Work out the finished part from the listing and answer in its coordinate system (mm). Coordinates: 2 decimals unless noted, no trailing zeros. Loops run counter-clockwise (first coordinate to the right, second up) from the corner with the lowest first, then second, coordinate; pieces in that order, holes last. Notation, with made-up numbers: (-25, -8.75) - (1, -8.75) arc R21 ccw to (1, 21.25) - close; hole circle Ø7 at (-28, 4.25). An arc over 180 degrees is marked (long way). Write each question's results on one line, items separated by ' | '. Start each with the question number.
1. Find the intervals of material crossed by line 1 along X through (y, z) = (2, 2.75); line 2 along Y through (x, z) = (-1.5, 4.1); line 3 along X through (y, z) = (-1.75, 0.8), in increasing order. Write a range as [from, to].
2. Each of these flat-tipped pins is pushed along its axis until it touches: P1, Ø1.5, axis at x = -3, z = 1, coming from the -Y side; P2, Ø2, axis at y = 0.5, z = 2.5, coming from the +X side (3 decimals); P3, Ø3, axis at y = 0, z = 2, coming from the -X side (3 decimals); P4, Ø4, axis at x = 0, y = 0, coming from the -Z side. Where does it stop, or does it pass through?
3. Determine the mould class of faces 1 (the flat face through (3.221, -1.895, 2.761)), 2 (the conical face through (-1.978, -3.406, 5.546)), 3 (the flat face through (0, 3.737, 3)), 4 (the cylindrical face through (-0.54, -2.44, 2.76)) for opening direction X: released by +X, released by -X, zero draft, split by the parting line, or undercut.
4. A cutting plane is placed at A-A on z = 3.9. Determine the outline of the cut face in (x, y) (1 decimal).
from build123d import *

# Parameters (mm, degrees)
SKETCH1_R          = 2.5
BOSS_EXTRUDE_DEPTH = 5.6
SKETCH2_OUTSIDE_W  = 296.81
SKETCH2_OUTSIDE_H  = 295.654
SKETCH2_OUTSIDE_R  = 3.736899617
CUT_EXTRUDE1_DEPTH = 38
CUT_EXTRUDE1_DRAFT = -75
SKETCH3_OUTSIDE_W  = 296.81
SKETCH3_OUTSIDE_H  = 295.654
SKETCH3_OUTSIDE_R  = 3.736899617
CUT_EXTRUDE2_DEPTH = 38
CUT_EXTRUDE2_DRAFT = -75
CHAMFER1_SIZE      = 0.2


with BuildPart() as part:
    # Sketch1 → Boss-Extrude (new body)
    with BuildSketch(Plane.XY):
        Polygon((2.1575, 3.736899617), (-2.1575, 3.736899617), (-4.315, 0), (-2.1575, -3.736899617), (2.1575, -3.736899617), (4.315, 0), align=None)
        Circle(SKETCH1_R, mode=Mode.SUBTRACT)
    extrude(amount=BOSS_EXTRUDE_DEPTH)


with BuildPart() as cut_extrude1_tool:
    # Sketch2 outside → Cut-Extrude1 (with draft: the straight prism first)
    with BuildSketch(Plane(origin=(0, 0, 0), x_dir=(-1, 0, 0), z_dir=(0, 0, -1))):
        Rectangle(SKETCH2_OUTSIDE_W, SKETCH2_OUTSIDE_H)
        Circle(SKETCH2_OUTSIDE_R, mode=Mode.SUBTRACT)
    extrude(amount=-CUT_EXTRUDE1_DEPTH)
    # Cut-Extrude1: the draft: its side faces are tilted about the plane it starts from
    cut_extrude1_sides = [cut_extrude1_tool.faces().sort_by_distance(p)[0] for p in [
        (0, -147.827, 19),
        (-148.405, 0, 19),
        (0, 147.827, 19),
        (148.405, 0, 19),
        (3.736899617, 0, 19),
    ]]
    draft(cut_extrude1_sides, Plane(origin=(0, 0, 0), x_dir=(-1, 0, 0), z_dir=(0, 0, -1)), CUT_EXTRUDE1_DRAFT)


with BuildPart() as part_1:
    add(part.part)

    # Cut-Extrude1: cut by cut_extrude1_tool
    add(cut_extrude1_tool.part, mode=Mode.SUBTRACT)


with BuildPart() as cut_extrude2_tool:
    # Sketch3 outside → Cut-Extrude2 (with draft: the straight prism first)
    with BuildSketch(Plane.XY.offset(5.6)):
        Rectangle(SKETCH3_OUTSIDE_W, SKETCH3_OUTSIDE_H)
        Circle(SKETCH3_OUTSIDE_R, mode=Mode.SUBTRACT)
    extrude(amount=-CUT_EXTRUDE2_DEPTH)
    # Cut-Extrude2: the draft: its side faces are tilted about the plane it starts from
    cut_extrude2_sides = [cut_extrude2_tool.faces().sort_by_distance(p)[0] for p in [
        (0, -147.827, -13.4),
        (148.405, 0, -13.4),
        (0, 147.827, -13.4),
        (-148.405, 0, -13.4),
        (-3.736899617, 0, -13.4),
    ]]
    draft(cut_extrude2_sides, Plane.XY.offset(5.6), CUT_EXTRUDE2_DRAFT)


with BuildPart() as part_2:
    add(part_1.part)

    # Cut-Extrude2: cut by cut_extrude2_tool
    add(cut_extrude2_tool.part, mode=Mode.SUBTRACT)

    # Chamfer1
    chamfer1_edges = [part_2.edges().sort_by_distance(p)[0] for p in [
        (-2.5, 0, 0),
        (-2.5, 0, 5.6),
    ]]
    chamfer(chamfer1_edges, length=CHAMFER1_SIZE)


solid = part_2.part
Values:
1) line 1: [-3.16, -1.5], [1.5, 3.16] | line 2: [-3.74, -2], [2, 3.74] | line 3: [-3.3, -1.79], [1.79, 3.3]
2) P1: y = -3.58 | P2: x = 4.315 | P3: x = -4.315 | P4: through
3) face 1: released by +X | face 2: released by -X | face 3: zero draft | face 4: undercut
4) outline: (-4.3, 0) - (-2.2, -3.7) - (2.2, -3.7) - (4.3, 0) - (2.2, 3.7) - (-2.2, 3.7) - close; hole circle Ø5 at (0, 0)
